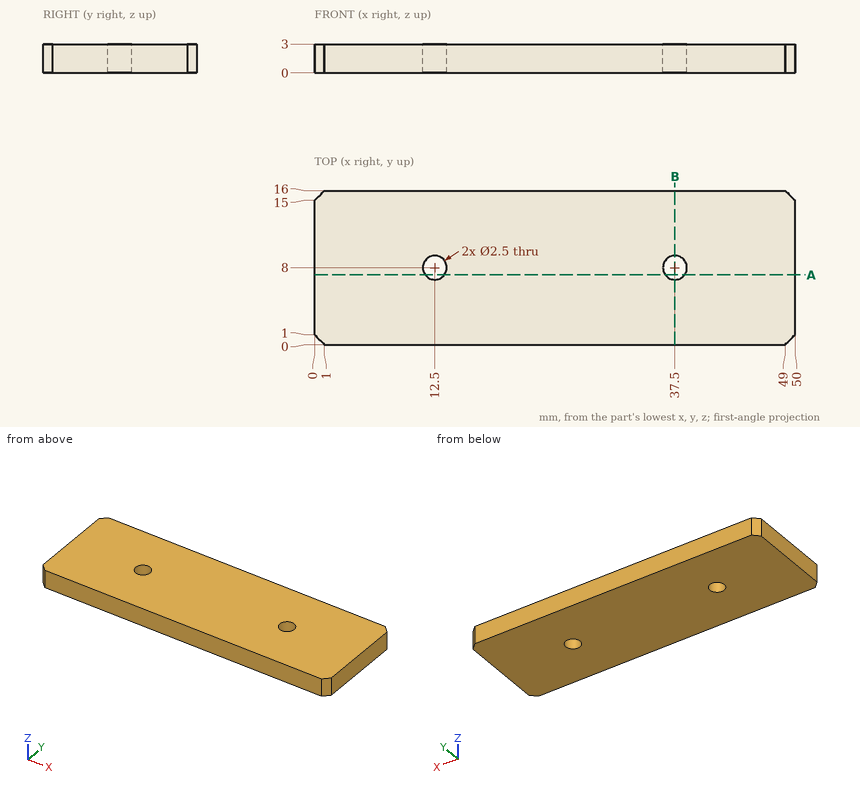
Geometry check sheet. Reference: drawing and pictorial views, mm from the part's lowest x, y, z. Coordinates: 2 decimals unless noted, no trailing zeros. Order: outer loops, then holes, each group sorted by start corner. A loop starts at its lowest first (then second) coordinate and runs counter-clockwise, first axis right, second up. Notation, with made-up numbers: (-23.75, 26) -> (10.25, 26) arc R21 ccw to (10.25, 56) -> close; hole circle Ø9 at (-11, -7.5). An arc over 180 degrees is marked (long way). Write item = value, one per line. Start each with the question number.
1) Material ranges on L1, parallel to Y at x = 37.5, z = 2; L2, parallel to X at y = 8.75, z = 0.6; L3, parallel to Y at x = 11.5, z = 1.6, recorded low to high.
2) Cross-section at A-A (y = 7.25). Enter the section's corners in (x, z), then the cut area to 3 significant figures.
3) Cross-section at B-B (x = 37.5). Enter the section's corners in (y, z), then the cut area to 3 significant figures.
Ans:
q1.L1 = 0 to 6.75, 9.25 to 16
q1.L2 = 0 to 11.5, 13.5 to 36.5, 38.5 to 50
q1.L3 = 0 to 7.25, 8.75 to 16
q2.outline = (0, 0) -> (11.5, 0) -> (11.5, 3) -> (0, 3) -> close; (13.5, 0) -> (36.5, 0) -> (36.5, 3) -> (13.5, 3) -> close; (38.5, 0) -> (50, 0) -> (50, 3) -> (38.5, 3) -> close
q2.area = 138 mm²
q3.outline = (0, 0) -> (6.75, 0) -> (6.75, 3) -> (0, 3) -> close; (9.25, 0) -> (16, 0) -> (16, 3) -> (9.25, 3) -> close
q3.area = 40.5 mm²
